Input: part model. Units: mm. Frame: model coordinates. Coordinates: 2 decimals unless noted, no trailing zeros. Loops run counter-clockwise (first coordinate to the right, second up) from the corner with the lowest first, then second, coordinate; pieces in that order, holes last.
Item 1: Section B-B on x = -51.5. Return loops of the section in (y, z).
Item 2: Section A-A on z = 2. Return loops of the section in (x, y).
Item 3: Contact query for flat-ended pins moving along their axis: P1, Ø5, axis at y = 396.5, z = 1.5, coming from the -X side; P2, Ø5, axis at y = 56, z = -3.5, coming from the +X side; P3, Ø12, axis at x = -135.5, y = 187.5, coming from the -Z side; P4, Ø5, axis at y = 303, z = 2, coming from the -X side. Output: stop coordinate, or through.
Item 4: Ray query, line 1 along X through (y, z) = (88.5, 3.5); line 2 along X through (y, z) = (285.5, -0.5). Return the intervals inside material, ascending.
Item 5: Section C-C on y = 261.5. Return loops of the section in (x, z).
```python
from build123d import *

# Parameters (mm, degrees)
BOSS_EXTRUDE1_DEPTH = 5


with BuildPart() as part:
    # Sketch1 → Boss-Extrude1 (new, symmetric)
    with BuildSketch(Plane.XY):
        Polygon((0, 130), (0, 500), (-20, 500), (-180, 20), (-180, 0), (-45, 0), align=None)
    extrude(amount=BOSS_EXTRUDE1_DEPTH, both=True)


solid = part.part
```
Results found:
1. outline: (0, -5) - (405.5, -5) - (405.5, 5) - (0, 5) - close
2. outline: (-180, 0) - (-45, 0) - (0, 130) - (0, 500) - (-20, 500) - (-180, 20) - close
3. P1: stops at x = -55.33
3. P2: stops at x = -24.75
3. P3: passes through
3. P4: stops at x = -86.5
4. line 1: x = -157.17 to -14.37
4. line 2: x = -91.5 to 0
5. outline: (-99.5, -5) - (0, -5) - (0, 5) - (-99.5, 5) - close
